For this review, use the dimensioned drawing (mm, ordinates from the lowest corner) and the shaded views. Give positions to 0.01 mm unless a question says otherwise; leave off trailing zeros. Write each loop counter-clockwise with the first axis right and the second up, starting at its lowest first coordinate (ties: lowest second). Pieces come first, ordered by that corner, then holes. Notation, with made-up numbers: M 19,60 L 23,60 A26 ccw 23,88 Z; hole C -17,81 d3. An arc over 180 degrees is marked long. Answer in a Markdown table with one row per item.
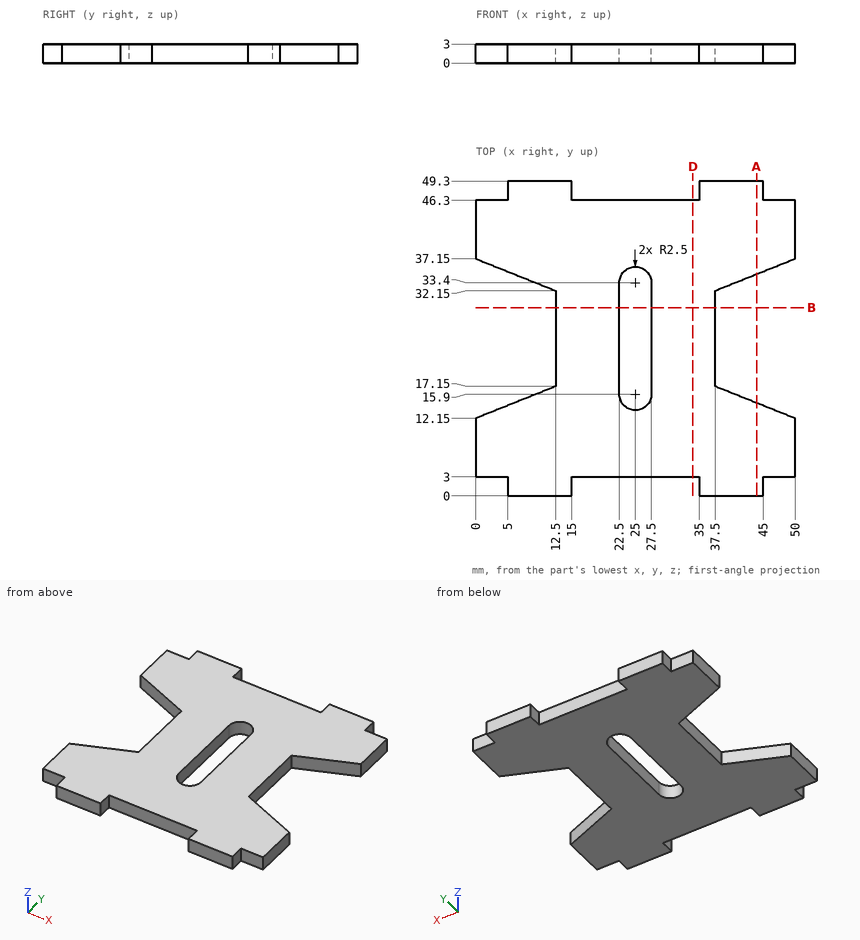
1) Add section B-B (y = 29.5). Write out the cut boundary in (x, z), and give its area (3 significant figures).
Geometry says:
| item | result |
|---|---|
| outline | M 12.5,0 L 22.5,0 L 22.5,3 L 12.5,3 Z; M 27.5,0 L 37.5,0 L 37.5,3 L 27.5,3 Z |
| area | 60.0 mm^2 |
2) Insertion check: P1, Ø5, axis at x = 27.5, y = 20, coming from the -Z side; P2, Ø1.5, axis at y = 48, z = 1, coming from the +X side; P3, Ø0.9, axis at y = 47.5, z = 1, coming from the -X side; P4, Ø0.9, axis at x = 24, z = 2, coming from the -Y side. Each pin has a flat end and moves straight along its axis. Give the tip position at first contact, or say it passes through.
Geometry says:
| item | result |
|---|---|
| P1 | z = 0 |
| P2 | x = 45 |
| P3 | x = 5 |
| P4 | y = 3 |
3) Add section D-D (x = 34). Write out the cut boundary in (y, z), and give its area (3 significant figures).
Geometry says:
| item | result |
|---|---|
| outline | M 3,0 L 46.3,0 L 46.3,3 L 3,3 Z |
| area | 130 mm^2 |
4) Add section A-A (x = 44). Write out the cut boundary in (y, z), and give its area (3 significant figures).
Geometry says:
| item | result |
|---|---|
| outline | M 0,0 L 14.55,0 L 14.55,3 L 0,3 Z; M 34.75,0 L 49.3,0 L 49.3,3 L 34.75,3 Z |
| area | 87.3 mm^2 |
5) To check wall thickness, follow probe 1 along X at (y, z) = (27, 2.1); probe 2 along Y at (x, z) = (15.5, 0.55); probe 3 along Y at (x, z) = (4, 2.1). State the ranges of each line that lie inside material, in increasing order. Write a range as [from, to].
Geometry says:
| item | result |
|---|---|
| probe 1 | [12.5, 22.5], [27.5, 37.5] |
| probe 2 | [3, 46.3] |
| probe 3 | [3, 13.75], [35.55, 46.3] |
